Could you check a few things on this drawing? It's one solid part, dimensions in mm from its lowest x, y, z. Give positions to 0.01 mm unless a question says otherwise; leave off trailing zeros. Loops run counter-clockwise (first coordinate to the right, second up) from the corner with the lowest first, then second, coordinate; pieces in that order, holes last. Notation, with made-up numbers: M 40.25,-8 L 88.25,-8 A14 ccw 88.25,3 Z; hole C 10,7.5 d11. An arc over 180 degrees is marked long. Answer as a JSON object with one key per item and string values.
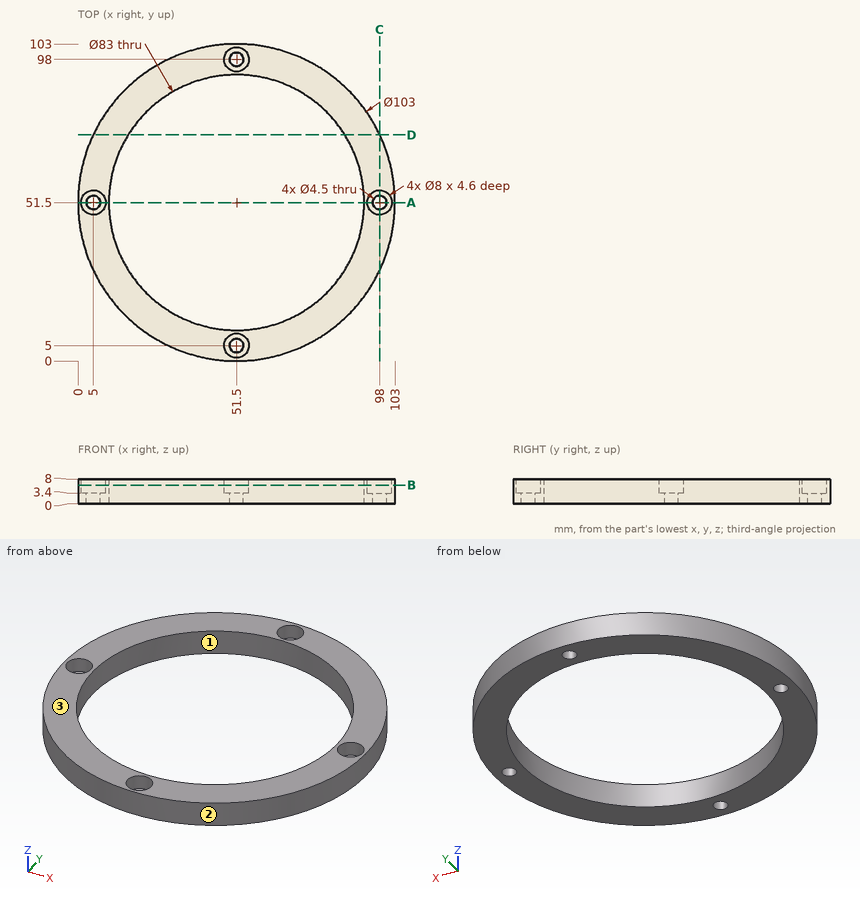
1) Will these pins go through, and if not, where does the flat tip stop? pin 1 Ø4 at (x, y) = (4.5, 52) entering from +Z; pin 2 Ø3.5 at (x, y) = (51.5, 5) entering from +Z; pin 3 Ø1.5 at (y, z) = (12.5, 4) entering from -X; pin 4 Ø1.5 at (y, z) = (35, 3.5) entering from -X.
Answer list:
{"pin 1": "z = 3.4", "pin 2": "through", "pin 3": "x = 17.02", "pin 4": "x = 2.47"}
2) Suppose I cut it at D-D, the plane y = 73.5. Write out the boundary of the cut face in (x, z), and give its area (3 significant figures).
Answer list:
{"outline": "M 4.94,0 L 16.31,0 L 16.31,8 L 4.94,8 Z; M 86.69,0 L 98.06,0 L 98.06,8 L 86.69,8 Z", "area": "182 mm^2"}
3) Suppose I cut it at C-C, the plane x = 98. Write out the boundary of the cut face in (y, z), and give its area (3 significant figures).
Answer list:
{"outline": "M 29.36,0 L 49.25,0 L 49.25,3.4 L 47.5,3.4 L 47.5,8 L 29.36,8 Z; M 53.75,0 L 73.64,0 L 73.64,8 L 55.5,8 L 55.5,3.4 L 53.75,3.4 Z", "area": "302 mm^2"}
4) Please list where these lines run through material, in increasing order: line 1 along Y through (x, z) = (51.5, 1.05); line 2 along X through (y, z) = (24, 7); line 3 along X through (y, z) = (98, 6). Write a range as from..to.
Answer list:
{"line 1": "0..2.75, 7.25..10, 93..95.75, 100.25..103", "line 2": "7.96..20.42, 82.58..95.04", "line 3": "29.36..47.5, 55.5..73.64"}
5) Suppose I cut it at B-B, the plane z = 6. Write out the boundary of the cut face in (x, y), and give its area (3 significant figures).
Answer list:
{"outline": "C 51.5,51.5 d103; hole C 5,51.5 d8; hole C 51.5,51.5 d83; hole C 51.5,5 d8; hole C 51.5,98 d8; hole C 98,51.5 d8", "area": "2,720 mm^2"}
6) Suppose I cut it at A-A, the plane y = 51.5. Write out the boundary of the cut face in (x, z).
Answer list:
{"outline": "M 0,0 L 2.75,0 L 2.75,3.4 L 1,3.4 L 1,8 L 0,8 Z; M 7.25,0 L 10,0 L 10,8 L 9,8 L 9,3.4 L 7.25,3.4 Z; M 93,0 L 95.75,0 L 95.75,3.4 L 94,3.4 L 94,8 L 93,8 Z; M 100.25,0 L 103,0 L 103,8 L 102,8 L 102,3.4 L 100.25,3.4 Z"}
7) If we mould it in two halves opening along X, with no side actions, what happens to the marked faces 1, 2 and 3? For each: +X half, -X half, draft (parallel to the pull), parting line (faces both ways), or undercut.
Answer list:
{"face 1": "undercut", "face 2": "parting line", "face 3": "draft"}
